The listing builds one solid part. Answer for the finished solid, in the listing's coordinates (mm). Face numbers are marked on the shaded views. Coordinates: 2 decimals unless noted, no trailing zeros. Loops run counter-clockwise (first coordinate to the right, second up) from the corner with the lowest first, then second, coordinate; pieces in that order, holes last. Notation, with made-up numbers: M -2.5,86 L 49.5,86 A15 ccw 49.5,114 Z; hole C -32.75,27.25 d2. An arc over 180 degrees is marked long. Answer in a Markdown table with one row per item. Add a question column.
from build123d import *

# Parameters (mm, degrees)
BOSS_EXTRUDE1_DEPTH = 9
CHAMFER1_SIZE       = 2
SKETCH2_R           = 3
CUT_EXTRUDE1_DEPTH  = 51.019996002


with BuildPart() as part:
    # Sketch1 → Boss-Extrude1 (new, symmetric)
    with BuildSketch(Plane.XY):
        Polygon((-16.5, -30), (-16.5, -27), (-13.5, -27), (-13.5, -24), (-10.5, -24), (-10.5, -21), (-7.5, -21), (-7.5, -18), (-4.5, -18), (-4.5, -15), (-1.5, -15), (-1.5, -12), (1.5, -12), (1.5, -15), (4.5, -15), (4.5, -18), (7.5, -18), (7.5, -21), (10.5, -21), (10.5, -24), (13.5, -24), (13.5, -27), (16.5, -27), (16.5, -30), (19.5, -30), (19.5, 30), (-19.5, 30), (-19.5, -30), align=None)
    extrude(amount=BOSS_EXTRUDE1_DEPTH, both=True)

    # Chamfer1
    chamfer1_edges = [part.edges().sort_by_distance(p)[0] for p in [
        (0, 30, 9),
        (0, 30, -9),
        (-19.5, 30, 0),
        (19.5, 30, 0),
    ]]
    chamfer(chamfer1_edges, length=CHAMFER1_SIZE)

    # Sketch2 → Cut-Extrude1 (cut, through all)
    with BuildSketch(Plane(origin=(19.5, 0, 0), x_dir=(0, 0, -1), z_dir=(1, 0, 0))):
        with Locations(Location((0, 23, 0), (0, 0, 90))):
            Circle(SKETCH2_R)
    extrude(amount=-CUT_EXTRUDE1_DEPTH, mode=Mode.SUBTRACT)

    # Sketch3 → Cut-Revolve1 (revolve, cut)
    with BuildSketch(Plane.XY, mode=Mode.PRIVATE) as cut_revolve1_sk:
        Polygon((0, 30), (6, 30), (6, 10), (0, 6.535898385), align=None)
    revolve(cut_revolve1_sk.sketch.rotate(Axis((0, 31.728134739, 0), (0, -1, 0)), 90), axis=Axis((0, 31.728134739, 0), (0, -1, 0)), mode=Mode.SUBTRACT)


solid = part.part
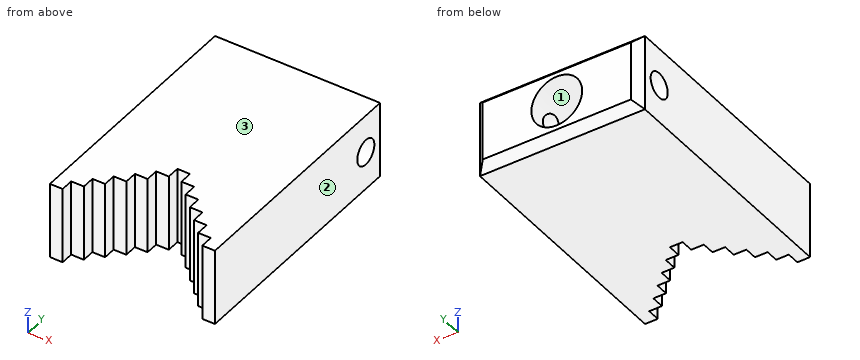
(1) The mould has two halves that part along X. Classify the marked faces 1, 2 and 3: released by +X, released by -X, zero draft, split by the parting line, or undercut.
(2) Straight lines are drawn through the part: line 1 (Y direction, x = 14, z = 0); line 2 (Z direction, x = -13, y = 23); line 3 (X direction, y = -14, z = -1.75). For each, find the intervals that lie inside material, in ascending order.
(3) Each of these flat-tipped pins is pushed along its axis until it touches: pin 1 (2.5 mm diameter, centred on x = -14.5, z = -4, fed in from -Y); pin 2 (1.5 mm diameter, centred on x = 4, z = -1.5, fed in from +Y); pin 3 (5 mm diameter, centred on x = 3.5, z = 2.5, fed in from -Y); pin 4 (3.5 mm diameter, centred on x = 15.5, z = 3, fed in from -Y). Where does it stop, or does it pass through?
(4) A cutting plane is placed at A-A (x = -9.5). Give the vertices of the cut face in (y, z).
(5) A cutting plane is placed at C-C (z = 0.75). State how many separate pieces and enclosed holes the cut face has, plus the area to 3 significant figures.
(6) A cutting plane is placed at B-B (y = 23). Give the vertices of the cut face in (x, z), plus the area to 3 significant figures.
Solved:
| question | item | result |
|---|---|---|
| 1 | face 1 | undercut |
| 1 | face 2 | released by +X |
| 1 | face 3 | zero draft |
| 2 | line 1 | y = -27 to 20, 26 to 30 |
| 2 | line 2 | z = -9 to -3, 3 to 9 |
| 2 | line 3 | x = -19.5 to -1.5, 1.5 to 19.5 |
| 3 | pin 1 | stops at y = -27 |
| 3 | pin 2 | stops at y = 9.44 |
| 3 | pin 3 | stops at y = -18 |
| 3 | pin 4 | stops at y = -30 |
| 4 | outline | M -21,-9 L 28,-9 L 30,-7 L 30,7 L 28,9 L -21,9 Z; hole C 23,0 d6 |
| 5 | separate pieces | 3 |
| 5 | enclosed holes | 0 |
| 5 | area | 1,600 mm² |
| 6 | outline | M -19.5,-9 L 19.5,-9 L 19.5,-3 L 5.2,-3 A6 cw -5.2,-3 L -19.5,-3 Z; M -19.5,3 L -5.2,3 A6 cw 5.2,3 L 19.5,3 L 19.5,9 L -19.5,9 Z |
| 6 | area | 424 mm² |
